The model under review builds one solid part; all positions refer to its coordinate system, in mm. Face numbers are marked on the shaded views. A direction names the side the tool comes from. Coordinates: 2 decimals unless noted, no trailing zeros. Write each loop counter-clockwise with the first axis right and the second up, starting at its lowest first coordinate (ties: lowest second). Pieces come first, ordered by that corner, then holes. Notation, with made-up numbers: M -11.5,-40 L 15.5,-40 A4 cw 15.5,-33 Z; hole C 63.25,21.5 d11. An arc over 180 degrees is marked long. Answer as a JSON object with one key per item and string values.
```python
from build123d import *

# Parameters (mm, degrees)
BRACKET_PROFILE_SKETCH_W  = 5
BRACKET_PROFILE_SKETCH_H  = 11
BRACKET_BODY_DEPTH        = 29
SADDLE_START              = -29
SKETCH1_4_R               = 6
SADDLE_STRAP_DEPTH        = 6
SQUARE_WINDOW_20X20_REACH = 86.865
SQUARE_WINDOW_SKETCH_R    = 10
CENTRE_GUSSET_DEPTH       = 5
CORNER_FILLET_R14_R       = 14
EDGE_NOTCH_REACH          = 86.865
EDGE_NOTCH_SKETCH_W       = 27
EDGE_NOTCH_SKETCH_H       = 26
NOTCH_FILLET_R6_R         = 6


with BuildPart() as part:
    # Bracket Profile Sketch → Bracket Body (new, symmetric)
    with BuildSketch(Plane.XY):
        with BuildLine():
            Line((0, -52), (0, 58))
            Line((0, 58), (-6, 58))
            ThreePointArc((-6, 58), (-20, 44), (-34, 58))
            Line((-34, 58), (-39, 58))
            ThreePointArc((-39, 58), (-26.892024376, 40.29406879), (-6, 45.154767421))
            Line((-6, 45.154767421), (-6, -52))
            Line((-6, -52), (0, -52))
        make_face()
        with Locations((-36.5, 63.5)):
            Rectangle(BRACKET_PROFILE_SKETCH_W, BRACKET_PROFILE_SKETCH_H)
    extrude(amount=BRACKET_BODY_DEPTH, both=True)

    # Sketch1_4 → Saddle Strap (add)
    with BuildSketch(Plane.XY.offset(SADDLE_START)):
        with BuildLine():
            ThreePointArc((38.203470161, 33.684210526), (34.310988843, 20), (38.203470161, 6.315789474))
            ThreePointArc((38.203470161, 6.315789474), (39.877604172, 1.709537694), (39.570464714, -3.181877796))
            Line((39.570464714, -3.181877796), (28.570464714, -43.181877796))
            ThreePointArc((28.570464714, -43.181877796), (24.27383896, -49.544174494), (17, -52))
            Line((17, -52), (0, -52))
            Line((0, -52), (0, 58))
            Line((0, 58), (30.413757643, 51.754734112))
            ThreePointArc((30.413757643, 51.754734112), (39.019735252, 44.750308934), (38.203470161, 33.684210526))
        make_face()
        with Locations((28, 40)):
            Circle(SKETCH1_4_R, mode=Mode.SUBTRACT)
        with Locations((28, 0)):
            Circle(SKETCH1_4_R, mode=Mode.SUBTRACT)
        with Locations((17, -40)):
            Circle(SKETCH1_4_R, mode=Mode.SUBTRACT)
    extrude(amount=SADDLE_STRAP_DEPTH)

    # Square Window Sketch → Square Window 20x20 (cut, up to next)
    with BuildSketch(Plane(origin=(0, 0, 0), x_dir=(0, 0, -1), z_dir=(1, 0, 0)), mode=Mode.PRIVATE) as square_window_20x20_sk1:
        with BuildLine():
            ThreePointArc((3, -52), (-8.283512569, -48.513096139), (-15.632572784, -39.268234411))
            Line((-15.632572784, -39.268234411), (-29, -5))
            Line((-29, -5), (-29, -52))
            Line((-29, -52), (3, -52))
        make_face()
    square_window_20x20_tool1 = extrude(square_window_20x20_sk1.sketch, amount=-SQUARE_WINDOW_20X20_REACH, mode=Mode.PRIVATE) & part.part
    # Square Window Sketch → Square Window 20x20 (cut, up to next)
    with BuildSketch(Plane(origin=(0, 0, 0), x_dir=(0, 0, -1), z_dir=(1, 0, 0)), mode=Mode.PRIVATE) as square_window_20x20_sk2:
        with Locations(Location((3, -32, 0), (0, 0, 90))):
            Circle(SQUARE_WINDOW_SKETCH_R)
    square_window_20x20_tool2 = extrude(square_window_20x20_sk2.sketch, amount=-SQUARE_WINDOW_20X20_REACH, mode=Mode.PRIVATE) & part.part
    add(square_window_20x20_tool1.solids().sort_by_distance((0, -37.269178, 21.871829))[0], mode=Mode.SUBTRACT)
    add(square_window_20x20_tool2.solids().sort_by_distance((0, -32, -3))[0], mode=Mode.SUBTRACT)

    # Centre Gusset Sketch → Centre Gusset (add, symmetric)
    with BuildSketch(Plane(origin=(0, 0, 0), x_dir=(1, 0, 0), z_dir=(0, 1, 0))):
        Polygon((0, 23), (0, -29), (22, 23), align=None)
    extrude(amount=CENTRE_GUSSET_DEPTH, both=True)

    # Corner Fillet R14
    corner_fillet_r14_edges = [part.edges().sort_by_distance(p)[0] for p in [
        (-6, 45.154767421, 0),
    ]]
    fillet(corner_fillet_r14_edges, radius=CORNER_FILLET_R14_R)

    # Edge Notch Sketch → Edge Notch (cut, up to next)
    with BuildSketch(Plane(origin=(0, 0, 0), x_dir=(0, 0, -1), z_dir=(1, 0, 0)), mode=Mode.PRIVATE) as edge_notch_sk1:
        with Locations((-3.5, 25)):
            Rectangle(EDGE_NOTCH_SKETCH_W, EDGE_NOTCH_SKETCH_H)
    edge_notch_tool1 = extrude(edge_notch_sk1.sketch, amount=-EDGE_NOTCH_REACH, mode=Mode.PRIVATE) & part.part
    add(edge_notch_tool1.solids().sort_by_distance((0, 25, 3.5))[0], mode=Mode.SUBTRACT)

    # Notch Fillet R6
    notch_fillet_r6_edges = [part.edges().sort_by_distance(p)[0] for p in [
        (-7.401923789, 38, 17),
        (-3, 12, -10),
        (-3, 12, 17),
        (-7.401923789, 38, -10),
    ]]
    fillet(notch_fillet_r6_edges, radius=NOTCH_FILLET_R6_R)


solid = part.part
```
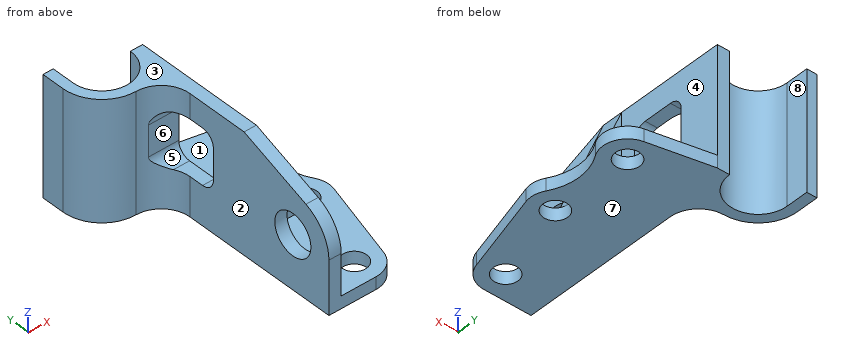
(1) Wall thickness on line 1 along Y through (x, z) = (28, -27); line 2 along Y through (x, z) = (14.5, -9); line 3 along Z through (x, y) = (17.5, -28): over which ranges is each line inside the solid? List them lowest first. Write a range as from..to.
Results list:
{"line 1": "-44.8..-6, 6..34, 46..52.25", "line 2": "-5..5", "line 3": "-29..-23"}
(2) Add section D-D on y = -15. Give the boundary of the cut face in (x, z), and give its area (3 significant figures).
Results list:
{"outline": "M -6,-29 L 36.32,-29 L 36.32,-23 L 0,-23 L 0,25.1 L -6,25.1 Z", "area": "543 mm²"}
(3) Add section B-B on x = 15. Give the boundary of the cut face in (y, z), and give its area (3 significant figures).
Results list:
{"outline": "M -52,-29 L -45.66,-29 L -45.66,-23 L -52,-23 Z; M -34.34,-29 L 54.92,-29 L 54.92,-23 L 5,-23 L 5,-6.45 L -5,-6.45 L -5,-23 L -34.34,-23 Z", "area": "739 mm²"}
(4) Add section A-A on y = 13.5. Give the boundary of the cut face in (x, z).
Results list:
{"outline": "M -6,-29 L 35.14,-29 L 35.14,-23 L 0,-23 L 0,-7.97 L -6,-7.97 Z; M -6,14.97 L 0,14.97 L 0,29 L -6,29 Z"}
(5) Draft analysis for pull direction Z (two halves, no side actions). For the marked faces 5, 6, 7 and 8, state which applies: released by +Z, released by -Z, zero draft, split by the parting line, or undercut.
Results list:
{"face 5": "undercut", "face 6": "undercut", "face 7": "released by -Z", "face 8": "zero draft"}
(6) Add section C-C on x = 7. Give the boundary of the cut face in (y, z), and give its area (3 significant figures).
Results list:
{"outline": "M -52,-29 L 56.56,-29 L 56.56,-23 L 5,-23 L 5,12.45 L -5,12.45 L -5,-23 L -52,-23 Z", "area": "1,010 mm²"}
(7) For pin 1 Ø24 at (x, z) = (14.5, 2.5) entering from -Y; pin 2 Ø6.5 at (x, z) = (8, 8.5) entering from +Y; pin 3 Ø19 at (x, y) = (17, -40) entering from +Z; pin 4 Ø9.5 at (x, y) = (28, 40) entering from +Z, all flat-tipped, find the tip position at first contact; note any pin that passes through.
Results list:
{"pin 1": "y = -5", "pin 2": "y = 5", "pin 3": "z = -23", "pin 4": "through"}
(8) For the marked faces 1, 2, 3 and 4, list the 3-axis set-ups (+Z, -Z, +X, -X, +Y, -Y) from which the entire face can be reached by the end or side of a thin tool; tool diameter is ignored.
Results list:
{"face 1": "+Z, +X", "face 2": "+Z, -Z, -X, -Y", "face 3": "+Z, +X, -X, +Y, -Y", "face 4": "+Z, +X, +Y"}
